from build123d import *

# Parameters (mm, degrees)
SKETCH2_W           = 12
SKETCH2_H           = 12
BOSS_EXTRUDE1_DEPTH = 8
CHAMFER1_SIZE       = 1
CUT_EXTRUDE1_DEPTH  = 3.5
CUT_EXTRUDE2_DEPTH  = 3.5


with BuildPart() as part:
    # Sketch1 → Revolve1 (revolve)
    with BuildSketch(Plane.XY, mode=Mode.PRIVATE) as revolve1_sk:
        Polygon((-41.365727984, 0), (28.134272016, 0), (28.134272016, 11), (14.134272016, 11), (14.134272016, 11.25), (8.134272016, 11.25), (8.134272016, 12), (4.134272016, 12), (4.134272016, 11), (-21.365727984, 11), (-21.365727984, 10), (-26.365727984, 10), (-26.365727984, 11), (-41.365727984, 11), align=None)
    revolve(revolve1_sk.sketch.rotate(Axis((-41.365727984, 0, 0), (1, 0, 0)), 90), axis=Axis((-41.365727984, 0, 0), (1, 0, 0)))

    # Sketch2 → Boss-Extrude1 (add)
    with BuildSketch(Plane.ZY.offset(41.365727984)):
        Rectangle(SKETCH2_W, SKETCH2_H)
    extrude(amount=BOSS_EXTRUDE1_DEPTH)

    # Chamfer1
    chamfer1_edges = [part.edges().sort_by_distance(p)[0] for p in [
        (-41.365727984, 0, -11),
        (28.134272016, 0, -11),
        (-45.365727984, -6, 6),
        (-45.365727984, 6, 6),
        (-45.365727984, 6, -6),
        (-45.365727984, -6, -6),
        (-49.365727984, 0, 6),
        (-49.365727984, 6, 0),
        (-49.365727984, 0, -6),
        (-49.365727984, -6, 0),
    ]]
    chamfer(chamfer1_edges, length=CHAMFER1_SIZE)

    # Sketch3 → Cut-Extrude1 (cut)
    with BuildSketch(Plane.XY.offset(11)):
        with BuildLine():
            Line((-15.865727984, 3), (-1.865727984, 3))
            ThreePointArc((-1.865727984, 3), (1.134272016, 0), (-1.865727984, -3))
            Line((-1.865727984, -3), (-15.865727984, -3))
            ThreePointArc((-15.865727984, -3), (-18.865727984, 0), (-15.865727984, 3))
        make_face()
    extrude(amount=-CUT_EXTRUDE1_DEPTH, mode=Mode.SUBTRACT)

    # Sketch4 → Cut-Extrude2 (cut)
    with BuildSketch(Plane.XY.offset(11)):
        with BuildLine():
            Line((-41.365727984, -2.5), (-31.365727984, -2.5))
            ThreePointArc((-31.365727984, -2.5), (-28.865727984, 0), (-31.365727984, 2.5))
            Line((-31.365727984, 2.5), (-41.365727984, 2.5))
            Line((-41.365727984, 2.5), (-41.365727984, -2.5))
        make_face()
    extrude(amount=-CUT_EXTRUDE2_DEPTH, mode=Mode.SUBTRACT)


solid = part.part
Can you work these out from the model? Positions are in its coordinate system, mm. A direction names the side the tool comes from. Coordinates: 2 decimals unless noted, no trailing zeros. Loops run counter-clockwise (first coordinate to the right, second up) from the corner with the lowest first, then second, coordinate; pieces in that order, holes last. Notation, with made-up numbers: M -39.75,-37.5 L -5.75,-37.5 A9 cw -5.75,-26.5 Z; hole C -21.75,78 d1. An arc over 180 degrees is marked long. Return JSON: item names as keys, results as strings. Group by question number.
Item 1: Imagine slicing it at C-C (x = 5.5). Please give me the cut outline in (y, z).
Item 2: On a 3-axis mill with a long thin cutter (end or side, diameter ignored), from which of +Z, -Z, +X, -X, +Y, -Y can I reach the whole of each face in a straight line? I mean faces 4 (the cylindrical face through (1.134, 0.066, 9.274)), 5 (the flat face through (-45, 0, 6)), 6 (the flat face through (-45, 0, -6)). Say none if no direction works.
Item 3: If I drill on L1, parallel to X at y = 7, z = 3.75; L2, parallel to Z at x = -24, y = 8; L3, parallel to X at y = -0.75, z = -10.5, over which ranges is the centre line in solid material (lowest first)? Write a range as from..to.
Item 4: Imagine slicing it at B-B (x = -13). Please give me the cut outline in (y, z), and give its area (3 significant figures).
Item 5: I'm going to push flat-ended pins straight in: pin 1 Ø3.5 at (x, z) = (-37.5, 9.5) entering from -Y; pin 2 Ø5.5 at (x, y) = (-33.5, -0.5) entering from +Z; pin 3 Ø3 at (x, y) = (-14.5, -7.5) entering from -Z; pin 4 Ø10 at (x, y) = (2, 2.5) entering from -Z. Where does each tip first touch, or does it pass through?
Item 6: Imagine slicing it at D-D (x = -30). Please give me the cut outline in (y, z), and give its area (3 significant figures).
Item 7: Thinking about a two-plate mould opening in Y: for faces 1 (the conical face through (-41.21, -0.41, -10.15)), 2 (the flat face through (8.134, -11, -3)), 3 (the flat face through (-36, 2.5, 9)), which applies, released by +Y, released by -Y, zero draft, split by the parting line, or undercut?
Verdict:
{
 "1": {"outline": "C 0,0 d24"},
 "2": {"face 4": "+Z", "face 5": "+Z, -X, +Y, -Y", "face 6": "-Z, -X, +Y, -Y"},
 "3": {"L1": "x = -41.37..28.13", "L2": "z = -6..6", "L3": "x = -40.84..-26.37, -21.37..27.61"},
 "4": {"outline": "M -3,7.5 L -3,10.58 A11 ccw long 3,10.58 L 3,7.5 Z", "area": "360 mm^2"},
 "5": {"pin 1": "stops at y = -7.81", "pin 2": "stops at z = 10.71", "pin 3": "stops at z = -9.22", "pin 4": "stops at z = -12"},
 "6": {"outline": "M -2.09,7.5 L -2.09,10.8 A11 ccw long 2.09,10.8 L 2.09,7.5 Z", "area": "366 mm^2"},
 "7": {"face 1": "split by the parting line", "face 2": "zero draft", "face 3": "undercut"}
}
